Study the drawing (mm; zero at the part's minimum x, y, z) and answer. A direction names the side the tool comes from. Give positions to 0.01 mm unless a question says otherwise; leave off trailing zeros. Write each loop counter-clockwise with the first axis right and the second up, starting at its lowest first coordinate (ties: lowest second). Pieces come first, ordered by that corner, then holes.
1) Given pin 1 Ø2.5 at (x, z) = (4.8, 3.3) entering from -Y; pin 2 Ø1 at (y, z) = (3.5, 5.5) entering from -X; pin 3 Ø1.5 at (x, z) = (6, 1.5) entering from +Y, each flat-ended and moving along its own axis, determine where each tip first touches the part or whether it passes through.
2) Straight lines are drawn through the part: probe 1 along Y at (x, z) = (14.5, 4.25); probe 2 along Y at (x, z) = (1.25, 4.75); probe 3 along Y at (x, z) = (13.75, 4). For each, find the intervals that lie inside material, in ascending order.
3) Find section C-C (x = 4.8). Determine the outline of the cut face in (y, z), plus the area to 3 significant figures.
4) Find section B-B (y = 3.5). Determine the outline of the cut face in (x, z).
5) Find section D-D (z = 5.75). Determine the outline of the cut face in (x, y).
6) A tool of negligible diameter and unlimited length cuts with its end or side. For the marked faces 1 and 2, from which of +Z, -Z, +X, -X, +Y, -Y can it reach the whole face along a straight path? Write none if from no direction.
7) Find section A-A (z = 3.3). Determine the outline of the cut face in (x, y).
8) Determine the mould class of the marked faces 3, 4 and 5 for opening direction Y: pulls with the +Y half, pulls with the -Y half, needs draft (parallel to the pull), parting line crosses it, or undercut.
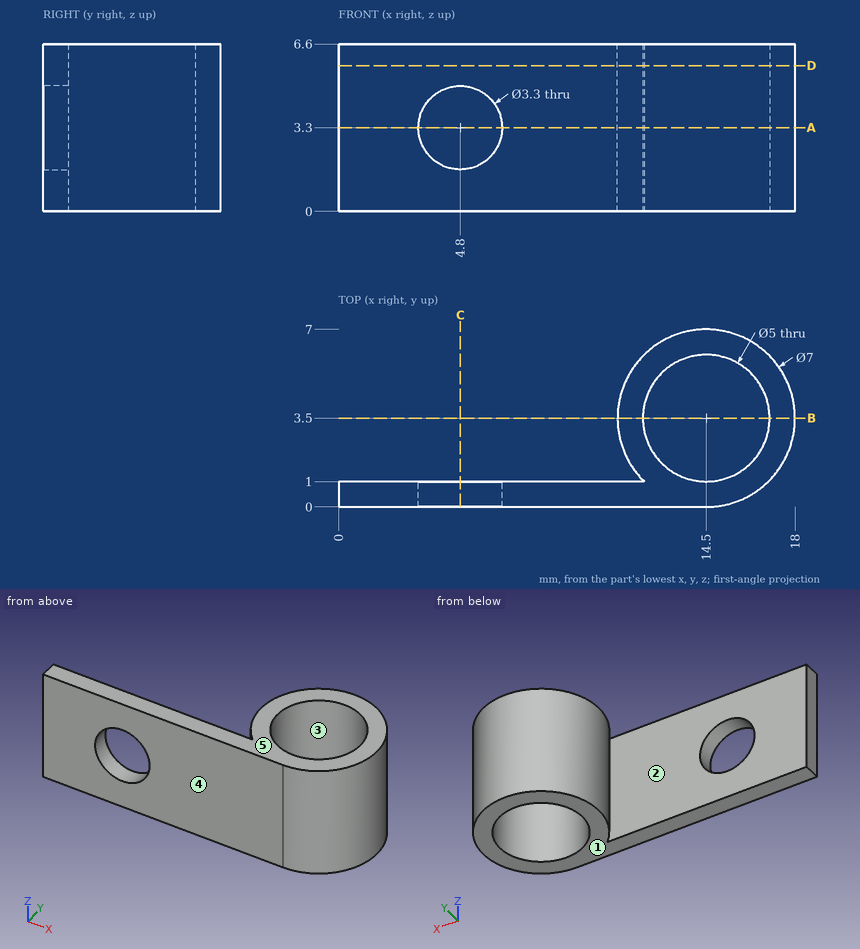
Results:
1. pin 1: passes through
1. pin 2: stops at x = 11
1. pin 3: stops at y = 1
2. probe 1: y = 0 to 1, 6 to 7
2. probe 2: y = 0 to 1
2. probe 3: y = 0 to 1.12, 5.88 to 6.92
3. outline: (0, 0) - (1, 0) - (1, 1.65) - (0, 1.65) - close; (0, 4.95) - (1, 4.95) - (1, 6.6) - (0, 6.6) - close
3. area: 3.30 mm2
4. outline: (11, 0) - (12, 0) - (12, 6.6) - (11, 6.6) - close; (17, 0) - (18, 0) - (18, 6.6) - (17, 6.6) - close
5. outline: (0, 0) - (14.5, 0) arc R3.5 ccw (long way) to (12.05, 1) - (0, 1) - close; hole circle Ø5 at (14.5, 3.5)
6. face 1: -Z, +X, -X, +Y, -Y
6. face 2: +Z, -Z, -X
7. outline: (0, 0) - (3.15, 0) - (3.15, 1) - (0, 1) - close; (6.45, 0) - (14.5, 0) arc R3.5 ccw (long way) to (12.05, 1) - (6.45, 1) - close; hole circle Ø5 at (14.5, 3.5)
8. face 3: undercut
8. face 4: pulls with the -Y half
8. face 5: needs draft
